```python
from build123d import *

# Parameters (mm, degrees)
BOSS_EXTRUDE1_DEPTH           = 480
COUNTERSINK_HOLE1_D           = 6
COUNTERSINK_HOLE1_CBORE_D     = 9.5
COUNTERSINK_HOLE1_CBORE_DEPTH = 8.5
LPATTERN1_COUNT               = 8
LPATTERN1_PITCH               = 60
CHAMFER1_SIZE                 = 1


with BuildPart() as part:
    # Sketch3 → Boss-Extrude1 (new body)
    with BuildSketch(Plane.XY):
        with BuildLine():
            Line((-10, -5), (10, -5))
            Line((10, -5), (10, 0))
            Line((10, 0), (7.7627417, 2.2372583))
            ThreePointArc((7.7627417, 2.2372583), (7.502614398, 2.626566319), (7.411269837, 3.085786438))
            Line((7.411269837, 3.085786438), (7.411269837, 4.851471863))
            ThreePointArc((7.411269837, 4.851471863), (7.502614398, 5.310691981), (7.7627417, 5.7))
            Line((7.7627417, 5.7), (10, 7.9372583))
            ThreePointArc((10, 7.9372583), (10.260127302, 8.326566319), (10.351471863, 8.785786438))
            Line((10.351471863, 8.785786438), (10.351471863, 10.551471863))
            ThreePointArc((10.351471863, 10.551471863), (10.260127302, 11.010691981), (10, 11.4))
            Line((10, 11.4), (8.751471863, 12.648528137))
            ThreePointArc((8.751471863, 12.648528137), (8.362163844, 12.908655439), (7.902943725, 13))
            Line((7.902943725, 13), (-7.902943725, 13))
            ThreePointArc((-7.902943725, 13), (-8.362163844, 12.908655439), (-8.751471863, 12.648528137))
            Line((-8.751471863, 12.648528137), (-10, 11.4))
            ThreePointArc((-10, 11.4), (-10.260127302, 11.010691981), (-10.351471863, 10.551471863))
            Line((-10.351471863, 10.551471863), (-10.351471863, 8.785786438))
            ThreePointArc((-10.351471863, 8.785786438), (-10.260127302, 8.326566319), (-10, 7.9372583))
            Line((-10, 7.9372583), (-7.7627417, 5.7))
            ThreePointArc((-7.7627417, 5.7), (-7.502614398, 5.310691981), (-7.411269837, 4.851471863))
            Line((-7.411269837, 4.851471863), (-7.411269837, 3.085786438))
            ThreePointArc((-7.411269837, 3.085786438), (-7.502614398, 2.626566319), (-7.7627417, 2.2372583))
            Line((-7.7627417, 2.2372583), (-10, 0))
            Line((-10, 0), (-10, -5))
        make_face()
    extrude(amount=-BOSS_EXTRUDE1_DEPTH)

    # Countersink Hole1 (through all)
    with Locations(Plane(origin=(0, 13, 0), x_dir=(-1, 0, 0), z_dir=(0, 1, 0))):
        with Locations((0, -30)):
            countersink_hole1 = CounterBoreHole(COUNTERSINK_HOLE1_D / 2, COUNTERSINK_HOLE1_CBORE_D / 2, COUNTERSINK_HOLE1_CBORE_DEPTH)

    # LPattern1: Countersink Hole1 ×8
    with Locations(*[(0, 0, -i * LPATTERN1_PITCH) for i in range(1, LPATTERN1_COUNT)]):
        add(countersink_hole1, mode=Mode.SUBTRACT)

    # Chamfer1
    chamfer1_edges = [part.edges().sort_by_distance(p)[0] for p in [
        (10, -5, -240),
        (-10, -5, -240),
    ]]
    chamfer(chamfer1_edges, length=CHAMFER1_SIZE)


solid = part.part
```
Input: part model. Units: mm. Frame: model coordinates. A direction names the side the tool comes from. Round coordinates to 2 decimals unless told otherwise and drop trailing zeros. Loops run counter-clockwise (first coordinate to the right, second up) from the corner with the lowest first, then second, coordinate; pieces in that order, holes last.
1) Pin query (flat end, axial travel): pin 1 (8 mm diameter, centred on y = -1.5, z = -357, fed in from +X). Return the tip coordinate at first contact, or that it passes through.
Ans:
pin 1: stops at x = 10
2) Pull-direction query (Z, two-part tool) for faces 3 (the flat face through (-3, 4.5, -451)), 4 (the flat face through (0, 4, 0)), 5 (the flat face through (0, -5, -237)); classes: released by +Z, released by -Z, zero draft, split by the parting line, or undercut.
Ans:
face 3: undercut
face 4: released by +Z
face 5: zero draft
3) Material intervals for line 1 (X direction, y = -2, z = -150); line 2 (X direction, y = 3.25, z = -384); line 3 (X direction, y = 2.25, z = -252.5), sorted ascending.
Ans:
line 1: x = -10 to -3, 3 to 10
line 2: x = -7.41 to 7.41
line 3: x = -7.75 to 7.75
4) Set-up query: faces 1 (the flat face through (-1, 4.5, -393)), 2 (the flat face through (0, 13, -237)). Return all of +Z, -Z, +X, -X, +Y, -Y with unobstructed straight access to the full face (end or side cutting, diameter ignored); none if empty.
Ans:
face 1: +Y
face 2: +Z, -Z, +X, -X, +Y
5) Section query A-A on z = -285.5. Return the cut outline in (x, y), plus the area to 3 significant figures.
Ans:
outline: (-10.35, 8.79) arc R1.2 ccw to (-10, 7.94) - (-7.76, 5.7) arc R1.2 cw to (-7.41, 4.85) - (-7.41, 3.09) arc R1.2 cw to (-7.76, 2.24) - (-10, 0) - (-10, -4) - (-9, -5) - (9, -5) - (10, -4) - (10, 0) - (7.76, 2.24) arc R1.2 cw to (7.41, 3.09) - (7.41, 4.85) arc R1.2 cw to (7.76, 5.7) - (10, 7.94) arc R1.2 ccw to (10.35, 8.79) - (10.35, 10.55) arc R1.2 ccw to (10, 11.4) - (8.75, 12.65) arc R1.2 ccw to (7.9, 13) - (-7.9, 13) arc R1.2 ccw to (-8.75, 12.65) - (-10, 11.4) arc R1.2 ccw to (-10.35, 10.55) - close
area: 331 mm2
